from build123d import *

# Parameters (mm, degrees)
EXTRUDE_1_DEPTH          = 12
CUT_EXTRUDE_1_DEPTH      = 65.815121692
CUT_EXTRUDE_1_DEPTH_BACK = 65.815121692
SKETCH_2_R               = 5.5


with BuildPart() as part:
    # 草图1 → 凸台-拉伸1 (new, symmetric)
    with BuildSketch(Plane(origin=(0, 0, 0), x_dir=(1, 0, 0), z_dir=(0, 1, 0))):
        with BuildLine():
            Line((8, -59), (4, -59))
            Line((4, -59), (4, -19.595917942))
            ThreePointArc((4, -19.595917942), (0, 20), (-4, -19.595917942))
            Line((-4, -19.595917942), (-4, -59))
            Line((-4, -59), (-8, -59))
            Line((-8, -59), (-8, -22.627416998))
            ThreePointArc((-8, -22.627416998), (0, 24), (8, -22.627416998))
            Line((8, -22.627416998), (8, -59))
        make_face()
    extrude(amount=EXTRUDE_1_DEPTH, both=True)

    # 草图2 → 切除-拉伸1 (cut, two sides: drawn at the far end of the back side and taken through both)
    with BuildSketch(Plane(origin=(0, 0, 0), x_dir=(0, 0, -1), z_dir=(1, 0, 0)).offset(-CUT_EXTRUDE_1_DEPTH_BACK)):
        with Locations((-39, 0)):
            Circle(SKETCH_2_R)
    extrude(amount=CUT_EXTRUDE_1_DEPTH + CUT_EXTRUDE_1_DEPTH_BACK, mode=Mode.SUBTRACT)


solid = part.part
Check sheet for the modelled part. Datum: model origin and axes. Units: mm. A direction names the side the tool comes from. Round coordinates to 2 decimals unless told otherwise and drop trailing zeros. Loops run counter-clockwise (first coordinate to the right, second up) from the corner with the lowest first, then second, coordinate; pieces in that order, holes last. Notation, with made-up numbers: (63.5, 73) -> (97.5, 73) arc R22 cw to (97.5, 89) -> close; hole circle Ø5 at (56.5, 69.5). An arc over 180 degrees is marked (long way). Put each result on its own line as item: value. Start each with the question number.
1. Scan lines: probe 1 along X at (y, z) = (6.5, 49.5); probe 2 along Z at (x, y) = (-6.8, 0); probe 3 along Z at (x, y) = (-5, 0). Record each from-to range of solid material in increasing order.
2. Section check C-C (x = 5). Enter the section's corners in (y, z), plus the area to 3 significant figures.
3. Section check D-D (z = 39). Enter the section's corners in (x, y).
4. Gauge pin test, flat ends, axial feed: pin 1 (5 mm diameter, centred on x = -2, z = 23.5, fed in from -Y); pin 2 (5 mm diameter, centred on y = -4.5, z = -7, fed in from -X); pin 3 (9 mm diameter, centred on y = 0, z = 39, fed in from -X); pin 4 (6 mm diameter, centred on x = 13.5, y = -1.5, fed in from -Z). Record the tip position at first contact, or that the pin passes through.
5. Section check B-B (y = 0). Enter the section's corners in (x, z).
6. Section check A-A (z = 0). Enter the section's corners in (x, y).
7. Draft check along X on faces 1 (the face through (8, 0, 45)), 2 (the face through (-4, 6, 39)), 3 (the face through (6, 0, 59)). Enter one of: +X half, -X half, draft (parallel to the pull), parting line (faces both ways), or undercut.
8. Access from +Z, -Z, +X, -X, +Y, -Y to the whole of each face (thin tool, end or side, straight path). Record for faces 4 (the face through (-8, 0, 45)), 5 (the face through (4, 3, 44)), 6 (the face through (-6, 0, 59)).
Findings:
1. probe 1: x = -8 to -4, 4 to 8
1. probe 2: z = -23.02 to -18.81, 18.81 to 33.5, 44.5 to 59
1. probe 3: z = -23.47 to -19.36, 19.36 to 33.5, 44.5 to 59
2. outline: (-12, -23.47) -> (12, -23.47) -> (12, -19.36) -> (-12, -19.36) -> close; (-12, 19.36) -> (12, 19.36) -> (12, 59) -> (-12, 59) -> close; hole circle Ø11 at (0, 39)
2. area: 955 mm^2
3. outline: (-8, -12) -> (-4, -12) -> (-4, -5.5) -> (-8, -5.5) -> close; (-8, 5.5) -> (-4, 5.5) -> (-4, 12) -> (-8, 12) -> close; (4, -12) -> (8, -12) -> (8, -5.5) -> (4, -5.5) -> close; (4, 5.5) -> (8, 5.5) -> (8, 12) -> (4, 12) -> close
4. pin 1: stops at y = -12
4. pin 2: stops at x = -23.57
4. pin 3: passes through
4. pin 4: stops at z = -21.58
5. outline: (-8, 22.63) arc R24 ccw (long way) to (8, 22.63) -> (8, 33.5) -> (4, 33.5) -> (4, 19.6) arc R20 cw (long way) to (-4, 19.6) -> (-4, 33.5) -> (-8, 33.5) -> close; (-8, 44.5) -> (-4, 44.5) -> (-4, 59) -> (-8, 59) -> close; (4, 44.5) -> (8, 44.5) -> (8, 59) -> (4, 59) -> close
6. outline: (-24, -12) -> (-20, -12) -> (-20, 12) -> (-24, 12) -> close; (20, -12) -> (24, -12) -> (24, 12) -> (20, 12) -> close
7. face 1: +X half
7. face 2: undercut
7. face 3: draft
8. face 4: +Z, -X, +Y, -Y
8. face 5: +Z, +Y, -Y
8. face 6: +Z, +X, -X, +Y, -Y
